Part model, mm, in its own coordinate system. A direction names the side the tool comes from. Round coordinates to 2 decimals unless told otherwise and drop trailing zeros. Write each loop counter-clockwise with the first axis right and the second up, starting at its lowest first coordinate (ties: lowest second). Pieces come first, ordered by that corner, then holes. Notation, with made-up numbers: M -26.5,-32 L 13.5,-32 A13 cw 13.5,-18 Z; hole C -26,62 d7. An arc over 180 degrees is marked long. Use one line per item in the form item = value. Start each with the question number.
Item 1: Probe L1, parallel to Y at x = 0, z = 81; L2, parallel to X at y = -1.5, z = -12. List the from-to ranges inside material, lowest first.
Item 2: Mould opens along Z. For faces 1 (the face through (1, -2.2, -87)), 2 (the face through (2.58, -4.05, 60.54)), 3 (the face through (0.35, 0.11, 71.96)) say: +Z half, -Z half, draft (parallel to the pull), parting line (faces both ways), or undercut.
Item 3: Flat gauge pins, fed straight in: pin 1 Ø1 at (y, z) = (1, 64.5) entering from +X; pin 2 Ø3.5 at (x, y) = (0, 0) entering from +Z; pin 3 Ø4 at (x, y) = (0, 0) entering from +Z. Where does each tip first touch, or does it go through?
Item 4: Which spindle directions (+Z, -Z, +X, -X, +Y, -Y) get a long thin tool onto all of the face, cutting with end or side? Do faces 4 (the face through (-1.08, -4.88, 74.23)), 5 (the face through (2.003, 0.631, -79.902)), 6 (the face through (2.58, -4.05, -55.56)), 7 (the face through (-2.003, 0.631, 79.902)). Say none if no direction does.
Item 5: Cut at A-A, the plane z = -42. Give the cut face in (x, y), then the cut area to 3 significant figures.
from build123d import *

# Parameters (mm, degrees)
SKETCH1_R             = 5
BOSS_EXTRUDE1_DEPTH   = 87
M5_TAPPED_HOLE1_D     = 4.2
M5_TAPPED_HOLE1_DEPTH = 14
M5_TAPPED_HOLE1_TIP   = 1.2618073
M5_TAPPED_HOLE2_D     = 4.2
M5_TAPPED_HOLE2_DEPTH = 14
M5_TAPPED_HOLE2_TIP   = 1.2618073
SKETCH10_W            = 1.1
SKETCH10_H            = 0.2


with BuildPart() as part:
    # Sketch1 → Boss-Extrude1 (new, symmetric)
    with BuildSketch(Plane.XY):
        Circle(SKETCH1_R)
    extrude(amount=BOSS_EXTRUDE1_DEPTH, both=True)

    # M5 Tapped Hole1
    with Locations(Plane(origin=(0, 0, -87), x_dir=(-1, 0, 0), z_dir=(0, 0, -1))):
        with Locations((0, 0)):
            Hole(M5_TAPPED_HOLE1_D / 2, depth=M5_TAPPED_HOLE1_DEPTH)
            with Locations((0, 0, -(M5_TAPPED_HOLE1_DEPTH + M5_TAPPED_HOLE1_TIP / 2))):  # 118° drill point
                Cone(0, M5_TAPPED_HOLE1_D / 2, M5_TAPPED_HOLE1_TIP, mode=Mode.SUBTRACT)

    # M5 Tapped Hole2
    with Locations(Plane.XY.offset(87)):
        with Locations((0, 0)):
            Hole(M5_TAPPED_HOLE2_D / 2, depth=M5_TAPPED_HOLE2_DEPTH)
            with Locations((0, 0, -(M5_TAPPED_HOLE2_DEPTH + M5_TAPPED_HOLE2_TIP / 2))):  # 118° drill point
                Cone(0, M5_TAPPED_HOLE2_D / 2, M5_TAPPED_HOLE2_TIP, mode=Mode.SUBTRACT)

    # Sketch10 → Cut-Revolve1 (revolve, cut)
    with BuildSketch(Plane(origin=(0, 0, 0), x_dir=(0, 0, -1), z_dir=(1, 0, 0)), mode=Mode.PRIVATE) as cut_revolve1_sk:
        with Locations((-60.55, 4.9)):
            Rectangle(SKETCH10_W, SKETCH10_H)
        with Locations((55.55, 4.9)):
            Rectangle(SKETCH10_W, SKETCH10_H)
    revolve(cut_revolve1_sk.sketch.rotate(Axis((0, 0, 87), (0, 0, -1)), 90), axis=Axis((0, 0, 87), (0, 0, -1)), mode=Mode.SUBTRACT)


solid = part.part
Model answer:
q1.L1 = -5 to -2.1, 2.1 to 5
q1.L2 = -4.77 to 4.77
q2.face_1 = -Z half
q2.face_2 = undercut
q2.face_3 = +Z half
q3.pin_1 = 4.97
q3.pin_2 = 72.79
q3.pin_3 = 72.94
q4.face_4 = +Z, -Z
q4.face_5 = -Z
q4.face_6 = none
q4.face_7 = +Z
q5.outline = C 0,0 d10
q5.area = 78.5 mm²
